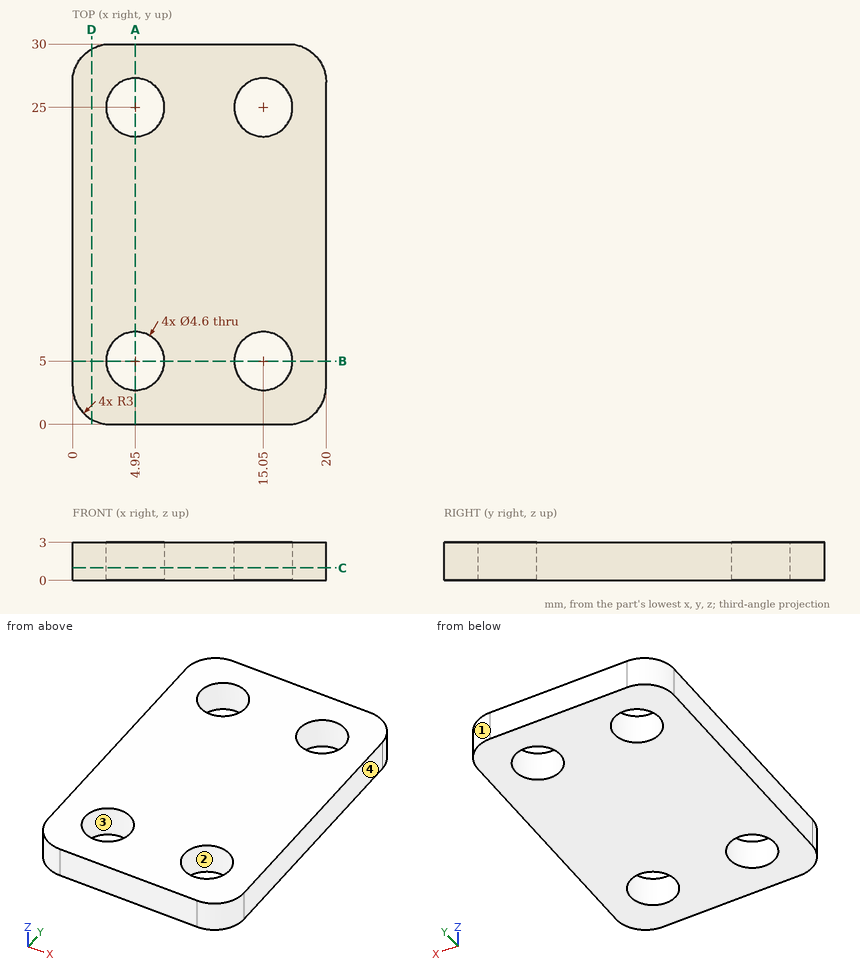
Print and shaded views of the part. All mm, measured from the part's lowest x, y and z. Coordinates: 2 decimals unless noted, no trailing zeros. Order: outer loops, then holes, each group sorted by start corner. A loop starts at its lowest first (then second) coordinate and runs counter-clockwise, first axis right, second up. Notation, with made-up numbers: (-39.75, -2.5) -> (3.25, -2.5) arc R23 ccw to (3.25, 7.5) -> close; hole circle Ø11 at (30.25, -16.75). An arc over 180 degrees is marked (long way). Answer as a JSON object with one key per item and string values. Group by question number.
1) Pull direction Y, two halves, no side cores. Call the marked faces 1, 2, 3 and 4: +Y half, -Y half, draft (parallel to the pull), parting line (faces both ways), or undercut.
2) Drill centre lines: L1, parallel to Y at x = 4.95, z = 1.1; L2, parallel to X at y = 23.75, z = 2.25; L3, parallel to Y at x = 5.75, z = 2.85. Where is each one in solid material? Low to high.
3) Cut at A-A, the plane x = 4.95. Write the cut outline in (y, z), then the cut area to 3 significant figures.
4) Cut at C-C, the plane z = 1. Write the cut outline in (x, y).
5) Cut at B-B, the plane y = 5. Write the cut outline in (x, z).
6) Cut at D-D, the plane x = 1.5. Write the cut outline in (y, z), then the cut area to 3 significant figures.
Check values:
{
 "1": {"face 1": "+Y half", "face 2": "undercut", "face 3": "undercut", "face 4": "draft"},
 "2": {"L1": "y = 0 to 2.7, 7.3 to 22.7, 27.3 to 30", "L2": "x = 0 to 3.02, 6.88 to 13.12, 16.98 to 20", "L3": "y = 0 to 2.84, 7.16 to 22.84, 27.16 to 30"},
 "3": {"outline": "(0, 0) -> (2.7, 0) -> (2.7, 3) -> (0, 3) -> close; (7.3, 0) -> (22.7, 0) -> (22.7, 3) -> (7.3, 3) -> close; (27.3, 0) -> (30, 0) -> (30, 3) -> (27.3, 3) -> close", "area": "62.4 mm²"},
 "4": {"outline": "(0, 3) arc R3 ccw to (3, 0) -> (17, 0) arc R3 ccw to (20, 3) -> (20, 27) arc R3 ccw to (17, 30) -> (3, 30) arc R3 ccw to (0, 27) -> close; hole circle Ø4.6 at (4.95, 5); hole circle Ø4.6 at (4.95, 25); hole circle Ø4.6 at (15.05, 5); hole circle Ø4.6 at (15.05, 25)"},
 "5": {"outline": "(0, 0) -> (2.65, 0) -> (2.65, 3) -> (0, 3) -> close; (7.25, 0) -> (12.75, 0) -> (12.75, 3) -> (7.25, 3) -> close; (17.35, 0) -> (20, 0) -> (20, 3) -> (17.35, 3) -> close"},
 "6": {"outline": "(0.4, 0) -> (29.6, 0) -> (29.6, 3) -> (0.4, 3) -> close", "area": "87.6 mm²"}
}
